Geometry: final body of the model. Coordinates: model frame, mm. Face numbers are marked on the shaded views. Coordinates: 2 decimals unless noted, no trailing zeros. Write each loop counter-clockwise with the first axis right and the second up, starting at its lowest first coordinate (ties: lowest second). Pieces come first, ordered by that corner, then holes. Notation, with made-up numbers: (-23.5, -10.5) - (13.5, -10.5) arc R22 cw to (13.5, -0.5) - close; hole circle Ø10 at (11, 89). An arc over 180 degrees is marked (long way). Put each result on its own line as item: value.
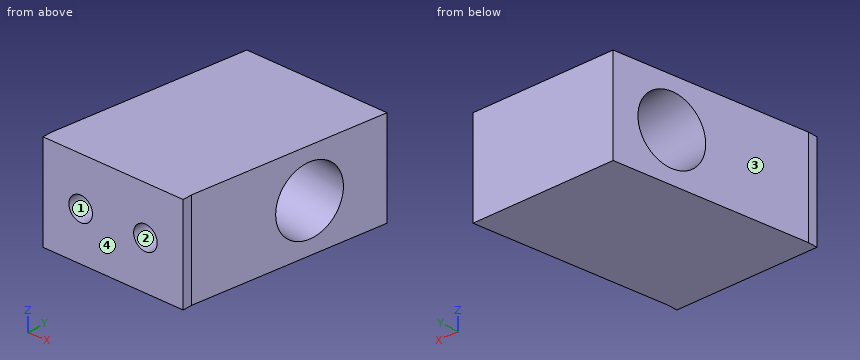
```python
from build123d import *

# Parameters (mm, degrees)
SKETCH_1_W          = 35
SKETCH_1_H          = 42
EXTRUDE_1_DEPTH     = 20
CUT_EXTRUDE_1_REACH = 39.577
CUT_EXTRUDE_2_REACH = 47.579
SKETCH_4_R          = 7
SKETCH_5_R          = 2.1
CUT_EXTRUDE_3_DEPTH = 14
SKETCH_6_R          = 2.5
CUT_EXTRUDE_4_DEPTH = 10


with BuildPart() as part:
    # 草图1 → 凸台-拉伸1 (new body)
    with BuildSketch(Plane.XY):
        with Locations((-4.192307692, -2.269230769)):
            Rectangle(SKETCH_1_W, SKETCH_1_H)
    extrude(amount=EXTRUDE_1_DEPTH)

    # 草图3 → 切除-拉伸1 (cut, up to next)
    with BuildSketch(Plane.XY.offset(20), mode=Mode.PRIVATE) as cut_extrude_1_sk1:
        Polygon((-21.692307692, 18.730769231), (-16.426307692, 18.730769231), (-21.692307692, -21.269230769), align=None)
    cut_extrude_1_tool1 = extrude(cut_extrude_1_sk1.sketch, amount=-CUT_EXTRUDE_1_REACH, mode=Mode.PRIVATE) & part.part
    # 草图3 → 切除-拉伸1 (cut, up to next)
    with BuildSketch(Plane.XY.offset(20), mode=Mode.PRIVATE) as cut_extrude_1_sk2:
        Polygon((13.307692308, 18.730769231), (8.041692308, -21.269230769), (8.041692308, -23.269230769), (13.307692308, -23.269230769), align=None)
    cut_extrude_1_tool2 = extrude(cut_extrude_1_sk2.sketch, amount=-CUT_EXTRUDE_1_REACH, mode=Mode.PRIVATE) & part.part
    add(cut_extrude_1_tool1.solids().sort_by_distance((-19.936974, 5.397436, 20))[0], mode=Mode.SUBTRACT)
    add(cut_extrude_1_tool2.solids().sort_by_distance((11.472571, -9.238928, 20))[0], mode=Mode.SUBTRACT)

    # 草图4 → 切除-拉伸2 (cut, up to next)
    with BuildSketch(Plane(origin=(-18.570357184, 2.444787523, 0), x_dir=(0, 0, 1), z_dir=(-0.9914451818173987, 0.13052375818626055, 0)), mode=Mode.PRIVATE) as cut_extrude_2_sk1:
        with Locations(Location((10, 4.307500918, 0), (0, 0, 270))):
            Circle(SKETCH_4_R)
    cut_extrude_2_tool1 = extrude(cut_extrude_2_sk1.sketch, amount=-CUT_EXTRUDE_2_REACH, mode=Mode.PRIVATE) & part.part
    add(cut_extrude_2_tool1.solids().sort_by_distance((-18.008126, 6.715439, 10))[0], mode=Mode.SUBTRACT)

    # 草图5 → 切除-拉伸3 (cut)
    with BuildSketch(Plane.XZ.offset(23.269230769)):
        with Locations((-13.692307692, 10)):
            Circle(SKETCH_5_R)
        with Locations((0.041692308, 10)):
            Circle(SKETCH_5_R)
    extrude(amount=-CUT_EXTRUDE_3_DEPTH, mode=Mode.SUBTRACT)

    # 草图6 → 切除-拉伸4 (cut)
    with BuildSketch(Plane.XZ.offset(23.269230769)):
        with Locations((-13.692307692, 10)):
            Circle(SKETCH_6_R)
        with Locations((0.041692308, 10)):
            Circle(SKETCH_6_R)
    extrude(amount=-CUT_EXTRUDE_4_DEPTH, mode=Mode.SUBTRACT)


solid = part.part
```
1. Section query B-B (y = -18). Return loops of the section in (x, z), then the cut area to 3 significant figures.
Answer below:
outline: (-21.26, 0) - (8.47, 0) - (8.47, 20) - (-21.26, 20) - close; hole circle Ø5 at (-13.69, 10); hole circle Ø5 at (0.04, 10)
area: 555 mm²
2. Section query C-C (z = 6.25). Return loops of the section in (x, y).
Answer below:
outline: (-21.69, -23.27) - (8.04, -23.27) - (8.04, -21.27) - (10.45, -2.99) - (-18.78, 0.86) - (-21.69, -21.27) - close; (-17.24, 12.58) - (11.99, 8.73) - (13.31, 18.73) - (-16.43, 18.73) - close
3. Ray query, probe 1 along Z at (x, y) = (8, 3); probe 2 along Y at (x, z) = (-8.5, 13.25); probe 3 along Y at (x, z) = (-13, 4.75). Return the intervals inside material, ascending. Write a range as from..to.
Answer below:
probe 1: z = 0..3.01, 16.99..20
probe 2: y = -23.27..-0.79, 11.72..18.73
probe 3: y = -23.27..1.39, 10.73..18.73
4. Mould query, pull axis X, two halves, no side actions, for the marked faces 1, 2, 3 and 4. Classes: +X half, -X half, draft (parallel to the pull), parting line (faces both ways), or undercut.
Answer below:
face 1: undercut
face 2: undercut
face 3: -X half
face 4: draft
5. Section query A-A (z = 11.25). Return loops of the section in (x, y), then the cut area to 3 significant figures.
Answer below:
outline: (-21.69, -23.27) - (-15.86, -23.27) - (-15.86, -13.27) - (-15.38, -13.27) - (-15.38, -9.27) - (-12, -9.27) - (-12, -13.27) - (-11.53, -13.27) - (-11.53, -23.27) - (-2.12, -23.27) - (-2.12, -13.27) - (-1.65, -13.27) - (-1.65, -9.27) - (1.73, -9.27) - (1.73, -13.27) - (2.21, -13.27) - (2.21, -23.27) - (8.04, -23.27) - (8.04, -21.27) - (10.32, -3.96) - (-18.91, -0.11) - (-21.69, -21.27) - close; (-17.11, 13.54) - (12.12, 9.7) - (13.31, 18.73) - (-16.43, 18.73) - close
area: 729 mm²
6. Pin query (flat end, axial travel): pin 1 Ø2 at (y, z) = (-11.5, 18) entering from -X; pin 2 Ø10 at (y, z) = (-6.5, 10.5) entering from -X; pin 3 Ø5 at (y, z) = (-10, 13.5) entering from +X. Return the tip coordinate at first contact, or that it passes through.
Answer below:
pin 1: stops at x = -20.54
pin 2: stops at x = -20.41
pin 3: stops at x = 9.85
